Check sheet for the drawn part. Datum: minimum x, y, z corner. Units: mm. A direction names the side the tool comes from. Coordinates: 2 decimals unless noted, no trailing zeros. Loops run counter-clockwise (first coordinate to the right, second up) from the corner with the lowest first, then second, coordinate; pieces in that order, holes last. Notation, with made-up numbers: (74.5, 39) - (125.5, 39) arc R25 ccw to (125.5, 71) - close; hole circle Ø9 at (87, -27.5). An arc over 180 degrees is marked (long way). Answer as a JSON object with one key per item and string values. Group by question number.
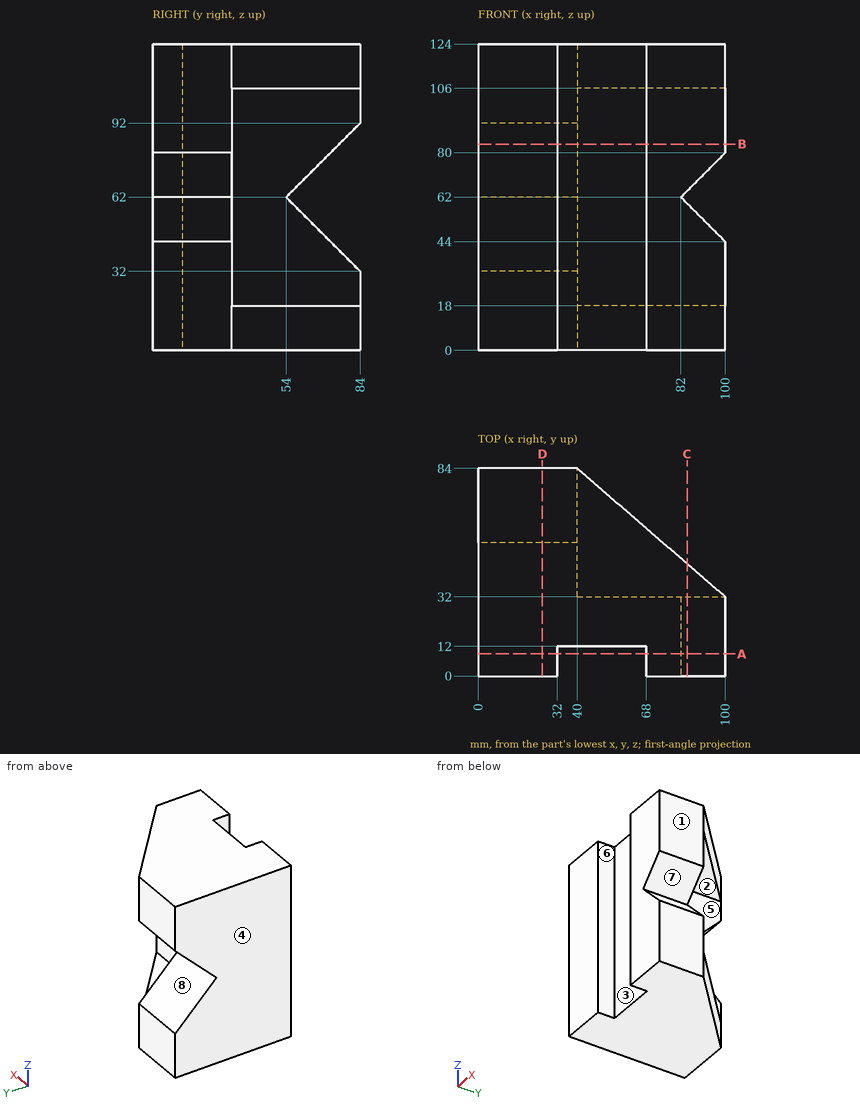
1. Sectioned sample at B-B on z = 83.5. Record the cut outline in (x, y), plus the area to 3 significant figures.
2. Sectioned sample at C-C on x = 84.5. Record the cut outline in (y, z), plus the area to 3 significant figures.
3. Material ranges on line 1 (Z direction, x = 42.5, y = 36); line 2 (Y direction, x = 62.5, z = 94); line 3 (X direction, y = 67.5, z = 37.5), recorded low to high.
4. Release check for a two-part mould opening along X. For the marked faces 1, 2, 3 and 4 record: released by +X, released by -X, zero draft, split by the parting line, or undercut.
5. Sectioned sample at A-A on y = 9. Record the cut outline in (x, z), plus the area to 3 significant figures.
6. Access from +Z, -Z, +X, -X, +Y, -Y to the whole of each face (thin tool, end or side, straight path). Record for the marked faces 5, 6, 7 and 8.
7. Sectioned sample at D-D on x = 26. Record the cut outline in (y, z), plus the area to 3 significant figures.
8. Gauge pin test, flat ends, axial feed: pin 1 (1 mm diameter, centred on y = 29.5, z = 78.5, fed in from +X); pin 2 (1.5 mm diameter, centred on y = 66.5, z = 104.5, fed in from +X). Record the tip position at first contact, or that the pin passes through.
Answers follow:
{
 "1": {"outline": "(0, 0) - (32, 0) - (32, 12) - (68, 12) - (68, 0) - (100, 0) - (100, 32) - (40, 32) - (40, 75.5) - (0, 75.5) - close", "area": "4,510 mm^2"},
 "2": {"outline": "(0, 0) - (45.43, 0) - (45.43, 18) - (32, 18) - (32, 59.5) - (0, 59.5) - close; (0, 64.5) - (32, 64.5) - (32, 106) - (45.43, 106) - (45.43, 124) - (0, 124) - close", "area": "4,290 mm^2"},
 "3": {"line 1": "z = 0 to 18, 106 to 124", "line 2": "y = 12 to 32", "line 3": "x = 0 to 40"},
 "4": {"face 1": "released by +X", "face 2": "zero draft", "face 3": "undercut", "face 4": "released by -X"},
 "5": {"outline": "(0, 0) - (32, 0) - (32, 124) - (0, 124) - close; (68, 0) - (100, 0) - (100, 44) - (82, 62) - (100, 80) - (100, 124) - (68, 124) - close", "area": "7,610 mm^2"},
 "6": {"face 5": "+X, +Y", "face 6": "+Z, -Z, -Y", "face 7": "+X, +Y, -Y", "face 8": "+X, -X, +Y"},
 "7": {"outline": "(0, 0) - (84, 0) - (84, 32) - (54, 62) - (84, 92) - (84, 124) - (0, 124) - close", "area": "9,520 mm^2"},
 "8": {"pin 1": "stops at x = 99", "pin 2": "stops at x = 40"}
}
